Work out the finished part from the listing and answer in its coordinate system (mm). A direction names the side the tool comes from. Round coordinates to 2 decimals unless told otherwise and drop trailing zeros. Write each loop counter-clockwise with the first axis right and the second up, starting at its lowest first coordinate (ties: lowest second). Pieces come first, ordered by that corner, then holes.
1. A tool of negligible diameter and unlimited length cuts with its end or side. For faces 1 (the face through (0, -25, 3)), 2 (the face through (-22, 0, 3)), from which of +Z, -Z, +X, -X, +Y, -Y can it reach the whole face along a straight path? Write none if from no direction.
2. Find section A-A (y = 13.5). Write down the section's boundary in (x, z), and give its area (3 significant figures).
3. Find section B-B (z = 121). Write down the section's boundary in (x, y).
4. Straight lines are drawn through the part: probe 1 along Y at (x, z) = (-4.5, 125); probe 2 along X at (y, z) = (-21.5, -135). For each, find the intervals that lie inside material, in ascending order.
5. Determine the mould class of faces 3 (the face through (-25, 0, 3)), 4 (the face through (0, 22, 3)), 5 (the face through (0, 25, 3)) for opening direction Y: pulls with the +Y half, pulls with the -Y half, needs draft (parallel to the pull), parting line crosses it, or undercut.
```python
from build123d import *

# Parameters (mm, degrees)
GB_6728_1986_050_X_50_X_3_1_DEPTH = 485


with BuildPart() as part:
    # Sketch1 → Gb／6728-1986方形空心型钢 050 X 50 X 3(1) (new body)
    with BuildSketch(Plane.YX.offset(-242.5)):
        with BuildLine():
            Line((-19, -25), (19, -25))
            ThreePointArc((19, -25), (23.242640687, -23.242640687), (25, -19))
            Line((25, -19), (25, 19))
            ThreePointArc((25, 19), (23.242640687, 23.242640687), (19, 25))
            Line((19, 25), (-19, 25))
            ThreePointArc((-19, 25), (-23.242640687, 23.242640687), (-25, 19))
            Line((-25, 19), (-25, -19))
            ThreePointArc((-25, -19), (-23.242640687, -23.242640687), (-19, -25))
        make_face()
        with BuildLine():
            Line((-19, -22), (19, -22))
            ThreePointArc((19, -22), (21.121320344, -21.121320344), (22, -19))
            Line((22, -19), (22, 19))
            ThreePointArc((22, 19), (21.121320344, 21.121320344), (19, 22))
            Line((19, 22), (-19, 22))
            ThreePointArc((-19, 22), (-21.121320344, 21.121320344), (-22, 19))
            Line((-22, 19), (-22, -19))
            ThreePointArc((-22, -19), (-21.121320344, -21.121320344), (-19, -22))
        make_face(mode=Mode.SUBTRACT)
    extrude(amount=GB_6728_1986_050_X_50_X_3_1_DEPTH)


solid = part.part
```
Worked answers:
1. face 1: +Z, -Z, +X, -X, -Y
1. face 2: +Z, -Z
2. outline: (-25, -242.5) - (-22, -242.5) - (-22, 242.5) - (-25, 242.5) - close; (22, -242.5) - (25, -242.5) - (25, 242.5) - (22, 242.5) - close
2. area: 2,910 mm2
3. outline: (-25, -19) arc R6 ccw to (-19, -25) - (19, -25) arc R6 ccw to (25, -19) - (25, 19) arc R6 ccw to (19, 25) - (-19, 25) arc R6 ccw to (-25, 19) - close; hole (-22, -19) arc R3 ccw to (-19, -22) - (19, -22) arc R3 ccw to (22, -19) - (22, 19) arc R3 ccw to (19, 22) - (-19, 22) arc R3 ccw to (-22, 19) - close
4. probe 1: y = -25 to -22, 22 to 25
4. probe 2: x = -24.45 to -20.66, 20.66 to 24.45
5. face 3: needs draft
5. face 4: undercut
5. face 5: pulls with the +Y half
